from build123d import *

# Parameters (mm, degrees)
BOSS_EXTRUDE1_DEPTH = 10


with BuildPart() as part:
    # Sketch2 → Boss-Extrude1 (new body)
    with BuildSketch(Plane.XY):
        with BuildLine():
            ThreePointArc((-369.098999305, 369.807855403), (-388.32594275, 360.628087401), (-406.481956169, 349.478976603))
            ThreePointArc((-406.481956169, 349.478976603), (-409.682668352, 332.093481456), (-392.297173205, 328.892769272))
            ThreePointArc((-392.297173205, 328.892769272), (-376.382642925, 338.665446638), (-359.529396201, 346.711909949))
            ThreePointArc((-359.529396201, 346.711909949), (-352.766225026, 363.044684228), (-369.098999305, 369.807855403))
        make_face()
        with BuildLine():
            ThreePointArc((-367.185078684, 365.188666312), (-385.937282785, 356.235559249), (-403.644999576, 345.361735137))
            ThreePointArc((-403.644999576, 345.361735137), (-405.565426886, 334.930438049), (-395.134129798, 333.010010739))
            ThreePointArc((-395.134129798, 333.010010739), (-378.77130289, 343.057974791), (-361.443316822, 351.33109904))
            ThreePointArc((-361.443316822, 351.33109904), (-357.385414117, 361.130763607), (-367.185078684, 365.188666312))
        make_face(mode=Mode.SUBTRACT)
    extrude(amount=BOSS_EXTRUDE1_DEPTH)


solid = part.part
Work out the finished part from the listing and answer in its coordinate system (mm). A direction names the side the tool comes from. Give positions to 0.01 mm unless a question says otherwise; leave off trailing zeros. Order: outer loops, then holes, each group sorted by start corner. A loop starts at its lowest first (then second) coordinate and runs counter-clockwise, first axis right, second up. Notation, with made-up numbers: M 81,24.25 L 95,24.25 A17 ccw 95,51.25 Z; hole C -38.75,88.25 d8. An arc over 180 degrees is marked long. Return JSON: item names as keys, results as strings.
Q1. Each of these flat-tipped pins is pushed along its axis until it touches: pin 1 (3 mm diameter, centred on x = -395.5, z = 4, fed in from -Y); pin 2 (5 mm diameter, centred on x = -360, y = 353, fed in from -Z); pin 3 (4 mm diameter, centred on y = 339, z = 6.5, fed in from +X); pin 4 (5 mm diameter, centred on y = 342.5, z = 6.5, fed in from -X). Where does it stop, or does it pass through?
Answer below:
{"pin 1": "stops at y = 326.92", "pin 2": "stops at z = 0", "pin 3": "stops at x = -371.94", "pin 4": "stops at x = -411.86"}
Q2. Find section D-D, the plane y = 368.5. Write down the section's boundary in (x, z), and give its area (3 significant figures).
Answer below:
{"outline": "M -372.18,0 L -357.15,0 L -357.15,10 L -372.18,10 Z", "area": "150 mm^2"}
Q3. Find section C-C, the plane y = 352. Write down the section's boundary in (x, z).
Answer below:
{"outline": "M -402.73,0 L -393.34,0 L -393.34,10 L -402.73,10 Z; M -360.18,0 L -353.49,0 L -353.49,10 L -360.18,10 Z"}
Q4. Find section B-B, the plane x = -363.5. Write down the section's boundary in (y, z), and give its area (3 significant figures).
Answer below:
{"outline": "M 345.01,0 L 350.46,0 L 350.46,10 L 345.01,10 Z; M 365.72,0 L 370.73,0 L 370.73,10 L 365.72,10 Z", "area": "105 mm^2"}
Q5. Find section A-A, the plane z = 2. Write down the section's boundary in (x, y) (3 decimals), and give its area (3 significant figures).
Answer below:
{"outline": "M -406.482,349.479 A12.5 ccw -392.297,328.893 A177.5 cw -359.529,346.712 A12.5 ccw -369.099,369.808 A202.5 ccw Z; hole M -403.645,345.362 A7.5 ccw -395.134,333.01 A182.5 cw -361.443,351.331 A7.5 ccw -367.185,365.189 A197.5 ccw Z", "area": "714 mm^2"}
Q6. The mould has two halves that part along Y. Classify faces 1 (the face through (-380, 342, 10)), 2 (the face through (-352.664, 362.79, 4.93)), 3 (the face through (-379.01, 342.93, 4.93)): pulls with the +Y half, pulls with the -Y half, needs draft (parallel to the pull), parting line crosses it, or undercut.
Answer below:
{"face 1": "needs draft", "face 2": "parting line crosses it", "face 3": "undercut"}
Q7. Find the intervals of material crossed by line 1 along Y through (x, z) = (-375.5, 3.75); line 2 along Y through (x, z) = (-360, 2.75); line 3 along X through (y, z) = (355.5, 4.5), in increasing order. Write a range as [from, to].
Answer below:
{"line 1": "y = [339.14, 344.79], [361.52, 367.03]", "line 2": "y = [346.52, 352.12], [364.39, 369.99]", "line 3": "x = [-397.21, -387.28], [-357.34, -352.12]"}
Q8. Which of the six approach directions +Z, -Z, +X, -X, +Y, -Y give full straight-line access (tool end or side, diameter ignored) to faces 4 (the face through (-385.681, 356.374, 4.93)), 5 (the face through (-376.61, 338.54, 4.93))?
Answer below:
{"face 4": "+Z, -Z", "face 5": "+Z, -Z, +X, -Y"}
